The drawing under review shows one solid part. Ordinate dimensions are in mm from its lowest x, y, z. Coordinates: 2 decimals unless noted, no trailing zeros. Order: outer loops, then holes, each group sorted by start corner. A loop starts at its lowest first (then second) coordinate and runs counter-clockwise, first axis right, second up.
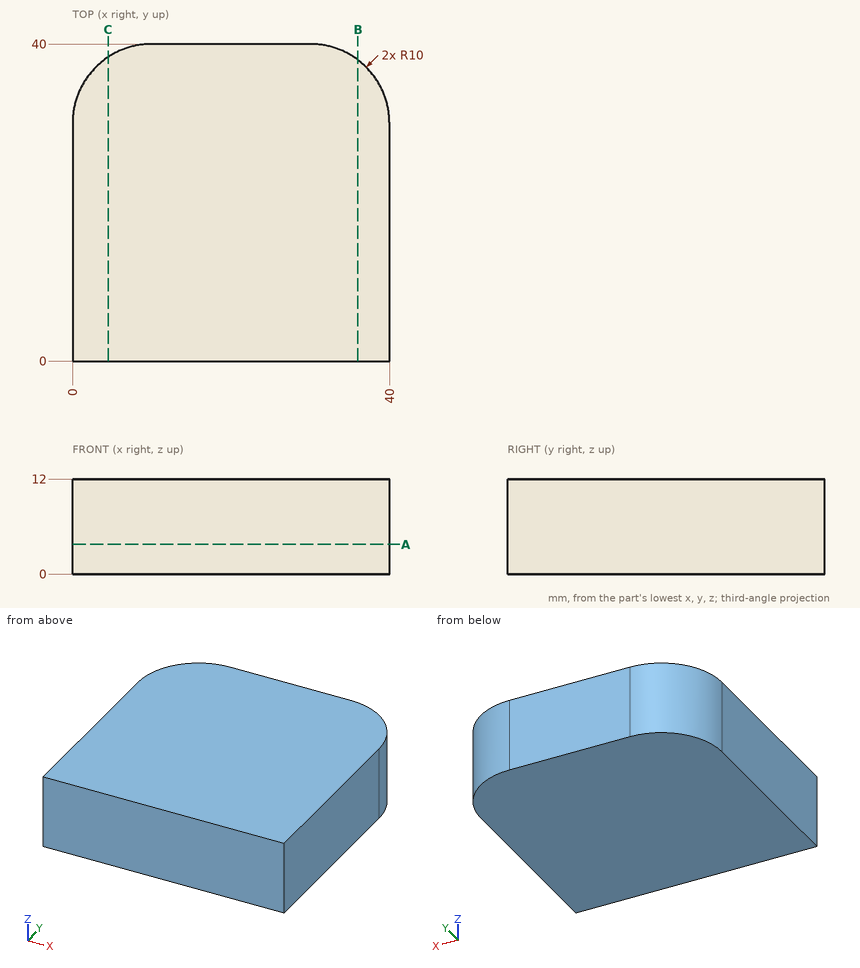
1. Take a section at A-A, the plane z = 3.75. Give the boundary of the cut face in (x, y).
Answer below:
outline: (0, 0) - (40, 0) - (40, 30) arc R10 ccw to (30, 40) - (10, 40) arc R10 ccw to (0, 30) - close
2. Take a section at C-C, the plane x = 4.5. Give the boundary of the cut face in (y, z).
Answer below:
outline: (0, 0) - (38.35, 0) - (38.35, 12) - (0, 12) - close
3. To check wall thickness, follow L1, parallel to Y at x = 5, z = 9; L2, parallel to Y at x = 4, z = 10.75; L3, parallel to X at y = 31, z = 8.75. State the ranges of each line that lie inside material, in increasing order.
Answer below:
L1: y = 0 to 38.66
L2: y = 0 to 38
L3: x = 0.05 to 39.95
4. Take a section at B-B, the plane x = 36. Give the boundary of the cut face in (y, z), plus the area to 3 significant figures.
Answer below:
outline: (0, 0) - (38, 0) - (38, 12) - (0, 12) - close
area: 456 mm2
5. Clearance check with a flat-ended pin moving along its axis: pin 1 Ø2 at (y, z) = (33.5, 7.5) entering from -X. State where the tip first meets the part, or that it passes through.
Answer below:
pin 1: stops at x = 0.32
